```python
from build123d import *

# Parameters (mm, degrees)
SKETCH_1_W                                        = 33
SKETCH_1_H                                        = 65
BOSS_EXTRUDE_1_DEPTH                              = 8
SKETCH_2_W                                        = 33
SKETCH_2_H                                        = 30
BOSS_EXTRUDE_2_DEPTH                              = 18
M3_HEX_SOCKET_CAP_SCREW_COUNTERBORE_1_D           = 3.4
M3_HEX_SOCKET_CAP_SCREW_COUNTERBORE_1_CBORE_D     = 6.5
M3_HEX_SOCKET_CAP_SCREW_COUNTERBORE_1_CBORE_DEPTH = 3
LINEAR_PATTERN_1_COUNT                            = 2
LINEAR_PATTERN_1_PITCH                            = 23
LINEAR_PATTERN_1_COUNT_DIR2                       = 2
LINEAR_PATTERN_1_PITCH_DIR2                       = 25
LINEAR_PATTERN_3_COUNT                            = 3
LINEAR_PATTERN_3_PITCH                            = 10
SKETCH_9_W                                        = 1.5
SKETCH_9_H                                        = 8
LINEAR_PATTERN_4_COUNT                            = 2
LINEAR_PATTERN_4_PITCH                            = 25
SKETCH_11_W                                       = 8
SKETCH_11_H                                       = 4
CUT_EXTRUDE_1_DEPTH                               = 18
LINEAR_PATTERN_5_COUNT                            = 2
LINEAR_PATTERN_5_PITCH                            = 20


with BuildPart() as part:
    # Sketch 1 → Boss-Extrude 1 (new body)
    with BuildSketch(Plane(origin=(0, 0, 0), x_dir=(0, 0, -1), z_dir=(1, 0, 0))):
        Rectangle(SKETCH_1_W, SKETCH_1_H)
    extrude(amount=BOSS_EXTRUDE_1_DEPTH)

    # Sketch 2 → Boss-Extrude 2 (add)
    with BuildSketch(Plane.ZY):
        with Locations((0, -17.5)):
            Rectangle(SKETCH_2_W, SKETCH_2_H)
    extrude(amount=BOSS_EXTRUDE_2_DEPTH)

    # M3 Hex Socket Cap Screw Counterbore 1 (through all)
    with Locations(Plane.ZY):
        with Locations((-11.5, 27.5)):
            m3_hex_socket_cap_screw_counterbore_1 = CounterBoreHole(M3_HEX_SOCKET_CAP_SCREW_COUNTERBORE_1_D / 2, M3_HEX_SOCKET_CAP_SCREW_COUNTERBORE_1_CBORE_D / 2, M3_HEX_SOCKET_CAP_SCREW_COUNTERBORE_1_CBORE_DEPTH)

    # Linear Pattern 1: M3 Hex Socket Cap Screw Counterbore 1 2 × 2
    with Locations(*[(0, -j * LINEAR_PATTERN_1_PITCH_DIR2, i * LINEAR_PATTERN_1_PITCH) for i in range(LINEAR_PATTERN_1_COUNT) for j in range(LINEAR_PATTERN_1_COUNT_DIR2) if (i, j) != (0, 0)]):
        add(m3_hex_socket_cap_screw_counterbore_1, mode=Mode.SUBTRACT)

    # Sketch 7 → M4 Tapped Hole 2 (revolve, cut)
    with BuildSketch(Plane(origin=(-18, -27.5, 0), x_dir=(0, 0, 1), z_dir=(0, 1, 0))):
        Polygon((0, 0), (0, 11.091420021), (1.65, 10.1), (1.65, 0), align=None)
    m4_tapped_hole_2 = revolve(axis=Axis((-24.35, -27.5, 0), (1, 0, 0)), mode=Mode.SUBTRACT)

    # Linear Pattern 3: M4 Tapped Hole 2 ×3
    with Locations(*[(0, i * LINEAR_PATTERN_3_PITCH, 0) for i in range(1, LINEAR_PATTERN_3_COUNT)]):
        add(m4_tapped_hole_2, mode=Mode.SUBTRACT)

    # Sketch 9 → Ø3.0 (3) Hole 1 (revolve, cut)
    with BuildSketch(Plane(origin=(0, 22.5, 11.5), x_dir=(0, 0, 1), z_dir=(0, 1, 0))):
        with Locations((0.75, 4)):
            Rectangle(SKETCH_9_W, SKETCH_9_H)
    f_3_0_3_hole_1 = revolve(axis=Axis((-6.35, 22.5, 11.5), (1, 0, 0)), mode=Mode.SUBTRACT)

    # Linear Pattern 4: Ø3.0 (3) Hole 1 ×2
    with Locations(*[(0, -i * LINEAR_PATTERN_4_PITCH, 0) for i in range(1, LINEAR_PATTERN_4_COUNT)]):
        add(f_3_0_3_hole_1, mode=Mode.SUBTRACT)

    # Sketch 11 → Cut-Extrude 1 (cut)
    with BuildSketch(Plane.ZY.offset(18)):
        with Locations((12.5, -4.5)):
            Rectangle(SKETCH_11_W, SKETCH_11_H)
    extrude(amount=-CUT_EXTRUDE_1_DEPTH, mode=Mode.SUBTRACT)

    # Sketch 12 → Ø4.0 (4) Hole 1 (revolve, cut)
    with BuildSketch(Plane(origin=(-18, -10, -10), x_dir=(0, 0, 1), z_dir=(0, 1, 0))):
        Polygon((0, 0), (0, 11.201721238), (2, 10), (2, 0), align=None)
    f_4_0_4_hole_1 = revolve(axis=Axis((-24.35, -10, -10), (1, 0, 0)), mode=Mode.SUBTRACT)

    # Linear Pattern 5: Ø4.0 (4) Hole 1 ×2
    with Locations(*[(0, 0, i * LINEAR_PATTERN_5_PITCH) for i in range(1, LINEAR_PATTERN_5_COUNT)]):
        add(f_4_0_4_hole_1, mode=Mode.SUBTRACT)


solid = part.part
```
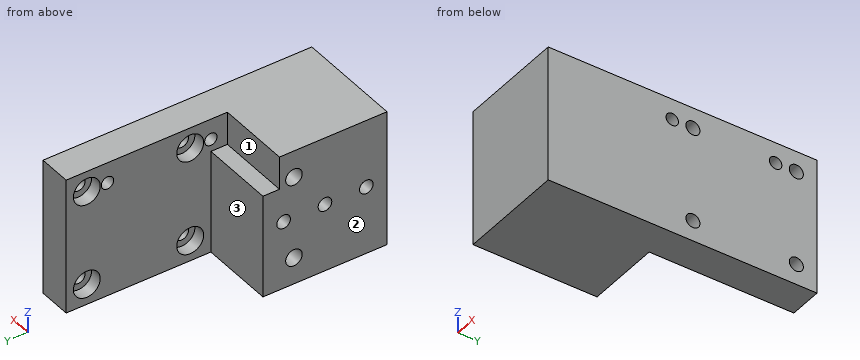
Model file for the job. Use its own axes, mm. Face numbers are marked on the shaded views. A direction names the side the tool comes from. Round coordinates to 2 decimals unless told otherwise and drop trailing zeros. Write each loop counter-clockwise with the first axis right and the second up, starting at its lowest first coordinate (ties: lowest second). Pieces come first, ordered by that corner, then holes. Notation, with made-up numbers: (26, 67) -> (42, 67) arc R5 ccw to (42, 71) -> close; hole circle Ø9 at (67, 74.25). An arc over 180 degrees is marked (long way). Answer as CSV lines item,"result".
1. Slice it at B-B, the plane x = 4. List the corners of the cut face in (y, z), plus the area to 3 significant figures.
Resolved:
outline,"(-32.5, -16.5) -> (32.5, -16.5) -> (32.5, 16.5) -> (-32.5, 16.5) -> close; hole circle Ø3 at (-2.5, 11.5); hole circle Ø3.4 at (2.5, -11.5); hole circle Ø3.4 at (2.5, 11.5); hole circle Ø3 at (22.5, 11.5); hole circle Ø3.4 at (27.5, -11.5); hole circle Ø3.4 at (27.5, 11.5)"
area,"2,090 mm²"
2. Drill centre lines: line 1 (Y direction, x = 1.3, z = -11.5); line 2 (Z direction, x = 2.25, y = -2.5); line 3 (Y direction, x = -12.75, z = -1). Where is each one in solid material? Low to high.
Resolved:
line 1,"-32.5 to -0.75, 5.75 to 24.25, 30.75 to 32.5"
line 2,"-16.5 to 10, 13 to 16.5"
line 3,"-32.5 to -28.81, -26.19 to -18.81, -16.19 to -8.81, -6.19 to -2.5"
3. Pin check, flat tips, straight feed: pin 1 Ø8 at (x, z) = (-4.5, 6) entering from +Y; pin 2 Ø3 at (y, z) = (-7.5, 0) entering from -X; pin 3 Ø2 at (y, z) = (29, -13) entering from -X; pin 4 Ø2.5 at (y, z) = (27.5, -11.5) entering from +X (3 decimals). Stop position of each tip, or through.
Resolved:
pin 1,"y = -2.5"
pin 2,"x = -7.81"
pin 3,"x = 3"
pin 4,"through"
4. Slice it at C-C, the plane z = 7. List the corners of the cut face in (x, y).
Resolved:
outline,"(-18, -32.5) -> (8, -32.5) -> (8, 32.5) -> (0, 32.5) -> (0, -2.5) -> (-18, -2.5) -> close"
5. Slice it at A-A, the plane y = 2.5. List the corners of the cut face in (x, z).
Resolved:
outline,"(0, -16.5) -> (8, -16.5) -> (8, -13.2) -> (3, -13.2) -> (3, -14.75) -> (0, -14.75) -> close; (0, -8.25) -> (3, -8.25) -> (3, -9.8) -> (8, -9.8) -> (8, 9.8) -> (3, 9.8) -> (3, 8.25) -> (0, 8.25) -> close; (0, 14.75) -> (3, 14.75) -> (3, 13.2) -> (8, 13.2) -> (8, 16.5) -> (0, 16.5) -> close"
6. Tool access for the marked faces 1, 2 and 3: list every direction of +Z, -Z, +X, -X, +Y, -Y with a clear straight run to the whole face (end or side of a thin tool).
Resolved:
face 1,"+Z, -X, +Y"
face 2,"+Z, -Z, -X, +Y, -Y"
face 3,"+Z, -Z, -X, +Y"
7. Slice it at D-D, the plane x = -1.75. List the corners of the cut face in (y, z), plus the area to 3 significant figures.
Resolved:
outline,"(-32.5, -16.5) -> (-2.5, -16.5) -> (-2.5, 8.5) -> (-6.5, 8.5) -> (-6.5, 16.5) -> (-32.5, 16.5) -> close"
area,"958 mm²"
